Can you work these out from the model? Positions are in its coordinate system, mm. Face numbers are marked on the shaded views. A direction names the side the tool comes from. Round coordinates to 2 decimals unless told otherwise and drop trailing zeros. Order: outer loops, then holes, each group sorted by start corner. A loop starts at its lowest first (then second) coordinate and runs counter-clockwise, first axis right, second up.
from build123d import *

# Parameters (mm, degrees)
EXTRUDE_1_DEPTH                = 5
HOLE_WIZARD_M4_1_D             = 3.3
EXTRUDE_3_DEPTH                = 10
HOLE_WIZARD_M4_1_2_D           = 4.5
HOLE_WIZARD_M4_1_2_CBORE_D     = 8
HOLE_WIZARD_M4_1_2_CBORE_DEPTH = 4.4
FILLET_1_R                     = 2
FILLET_2_R                     = 5


with BuildPart() as part:
    # 草图1 → 凸台-拉伸1 (new, symmetric)
    with BuildSketch(Plane(origin=(0, 0, 0), x_dir=(1, 0, 0), z_dir=(0, 1, 0))):
        Polygon((-12, -15), (48.355339059, -15), (13, 20.355339059), (-12, 20.355339059), align=None)
    extrude(amount=EXTRUDE_1_DEPTH, both=True)

    # Hole Wizard M4 _1 (through all)
    with Locations(Plane(origin=(0, -5, 0), x_dir=(-1, 0, 0), z_dir=(0, -1, 0))):
        with Locations((8, 2.67766953), (-2, 2.67766953)):
            Hole(HOLE_WIZARD_M4_1_D / 2)

    # 草图5 → 凸台-拉伸3 (add)
    with BuildSketch(Plane.XZ.offset(5)):
        Polygon((13.707106781, -10.455844123), (39.162950904, 15), (48.355339059, 15), (18.303300859, -15.0520382), align=None)
    extrude_3 = extrude(amount=EXTRUDE_3_DEPTH)

    # 镜向1: 凸台-拉伸3 across plane
    add(extrude_3.mirror(Plane.ZX))

    # Hole Wizard M4 _1 2 (through all)
    with Locations(Plane(origin=(12.081475452, 0, -12.081475452), x_dir=(0.7071067811865515, 0, 0.7071067811865436), z_dir=(-0.7071067811865436, 0, 0.7071067811865515))):
        with Locations((8.798989873, 10), (30.798989873, 10), (8.798989873, -10), (30.798989873, -10)):
            CounterBoreHole(HOLE_WIZARD_M4_1_2_D / 2, HOLE_WIZARD_M4_1_2_CBORE_D / 2, HOLE_WIZARD_M4_1_2_CBORE_DEPTH)

    # 圆角1
    fillet_1_edges = [part.edges().sort_by_distance(p)[0] for p in [
        (13.707106781, -10, -10.455844123),
        (13.707106781, 10, -10.455844123),
    ]]
    fillet(fillet_1_edges, radius=FILLET_1_R)

    # 圆角2
    fillet_2_edges = [part.edges().sort_by_distance(p)[0] for p in [
        (-12, 0, 15),
        (-12, 0, -20.355339059),
    ]]
    fillet(fillet_2_edges, radius=FILLET_2_R)


solid = part.part
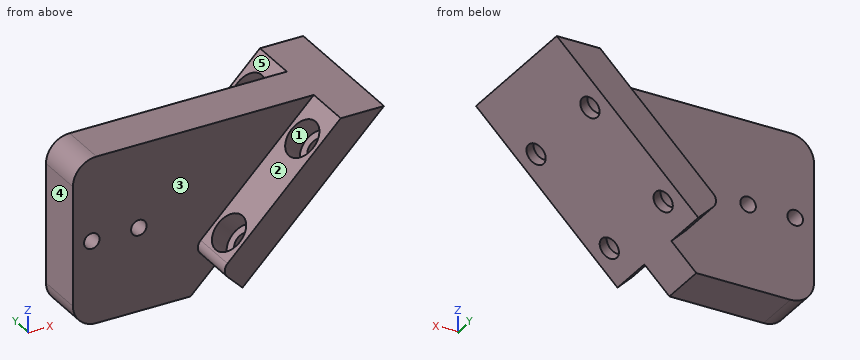
(1) I want a section at B-B, the plane y = -10.75. List the corners of the cut face in (x, z) for me, plus the area to 3 significant figures.
(2) Please list where these lines run through material, in increasing order: probe 1 along Z at (x, y) = (2, -0.5); probe 2 along Y at (x, z) = (10.5, 11); probe 3 along Z at (x, y) = (3, 3).
(3) I want a section at C-C, the plane x = 28. List the corners of the cut face in (y, z) for me, plus the area to 3 significant figures.
(4) If we mould it in two halves opening along Y, with no side actions, what happens to the marked faces 1, 2 and 3? For each: pulls with the +Y half, pulls with the -Y half, needs draft (parallel to the pull), parting line crosses it, or undercut.
(5) I want a section at A-A, the plane x = 2. List the corners of the cut face in (y, z) for me, plus the area to 3 significant figures.
(6) I want a section at D-D, the plane z = -18. List the corners of the cut face in (x, y) for me.
(7) On a 3-axis mill with a long thin cutter (end or side, diameter ignored), from which of +Z, -Z, +X, -X, +Y, -Y can I reach the whole of each face in a straight line? I mean the marked faces 4 and 5. Say none if no direction works.
(8) I'm going to push flat-ended pins straight in: pin 1 Ø2.5 at (x, z) = (-8, -2.68) entering from +Y; pin 2 Ø6 at (x, z) = (1, 6) entering from -Y; pin 3 Ø5 at (x, y) = (16, 8.5) entering from +Z; pin 4 Ø1.5 at (x, y) = (41.5, -7.5) entering from -Z. Where does each tip first touch, or does it pass through?
Ans:
1. outline: (15.12, -11.87) - (18.3, -15.05) - (21.4, -11.96) - (19.91, -10.47) - (18.64, -11.75) - (15.53, -8.64) - (15.12, -9.04) arc R2 ccw to start; (21.08, -3.08) - (24.19, -6.19) - (22.91, -7.47) - (24.4, -8.96) - (36.96, 3.6) - (35.47, 5.09) - (34.19, 3.81) - (31.08, 6.92) - close; (36.64, 12.47) - (39.75, 9.36) - (38.47, 8.09) - (39.96, 6.6) - (48.36, 15) - (39.16, 15) - close
1. area: 167 mm2
2. probe 1: z = -20.36 to -4.33, -1.03 to 15
2. probe 2: y = -5 to 5
2. probe 3: z = -20.36 to -3.99, -1.37 to 15
3. outline: (-15, -5.36) - (15, -5.36) - (15, 3.84) - (5, 3.84) - (5, 15) - (-5, 15) - (-5, 3.84) - (-15, 3.84) - close
3. area: 387 mm2
4. face 1: undercut
4. face 2: needs draft
4. face 3: pulls with the -Y half
5. outline: (-5, -20.36) - (5, -20.36) - (5, -4.33) - (-5, -4.33) - close; (-5, -1.03) - (5, -1.03) - (5, 15) - (-5, 15) - close
5. area: 321 mm2
6. outline: (-11.24, -5) - (15.36, -5) - (15.36, 5) - (-11.24, 5) - close
7. face 4: +Z, -Z, -X, +Y, -Y
7. face 5: +Z, -X, +Y
8. pin 1: passes through
8. pin 2: stops at y = -5
8. pin 3: stops at z = -6.95
8. pin 4: stops at z = 7.39
